```python
from build123d import *

# Parameters (mm, degrees)
SKETCH1_R           = 6
BOSS_EXTRUDE1_DEPTH = 91
SKETCH2_R           = 24.5
BOSS_EXTRUDE2_DEPTH = 4
SKETCH3_R           = 6
BOSS_EXTRUDE3_DEPTH = 3
BOSS_EXTRUDE4_DEPTH = 12
SKETCH5_R           = 6
BOSS_EXTRUDE5_DEPTH = 18
CHAMFER1_SIZE       = 0.9
SKETCH6_R           = 3
BOSS_EXTRUDE6_DEPTH = 20


with BuildPart() as part:
    # Sketch1 → Boss-Extrude1 (new body)
    with BuildSketch(Plane.XY):
        Circle(SKETCH1_R)
    extrude(amount=BOSS_EXTRUDE1_DEPTH)

    # Sketch2 → Boss-Extrude2 (add)
    with BuildSketch(Plane.XY.offset(91)):
        Circle(SKETCH2_R)
    extrude(amount=BOSS_EXTRUDE2_DEPTH)

    # Sketch3 → Boss-Extrude3 (add)
    with BuildSketch(Plane.XY.offset(95)):
        Circle(SKETCH3_R)
    extrude(amount=BOSS_EXTRUDE3_DEPTH)

    # Sketch4 → Boss-Extrude4 (add)
    with BuildSketch(Plane.XY.offset(98)):
        with BuildLine():
            Line((6, 5.291502622), (6, -5.291502622))
            ThreePointArc((6, -5.291502622), (0, -8), (-6, -5.291502622))
            Line((-6, -5.291502622), (-6, 5.291502622))
            ThreePointArc((-6, 5.291502622), (0, 8), (6, 5.291502622))
        make_face()
    extrude(amount=BOSS_EXTRUDE4_DEPTH)

    # Sketch5 → Boss-Extrude5 (add)
    with BuildSketch(Plane.XY.offset(110)):
        Circle(SKETCH5_R)
    extrude(amount=BOSS_EXTRUDE5_DEPTH)

    # Chamfer1
    chamfer1_edges = [part.edges().sort_by_distance(p)[0] for p in [
        (-6, 0, 0),
        (-6, 0, 128),
    ]]
    chamfer(chamfer1_edges, length=CHAMFER1_SIZE)

    # Sketch6 → Boss-Extrude6 (add)
    with BuildSketch(Plane.XY.offset(95)):
        with Locations((20, 0)):
            Circle(SKETCH6_R)
    extrude(amount=BOSS_EXTRUDE6_DEPTH)


solid = part.part
```
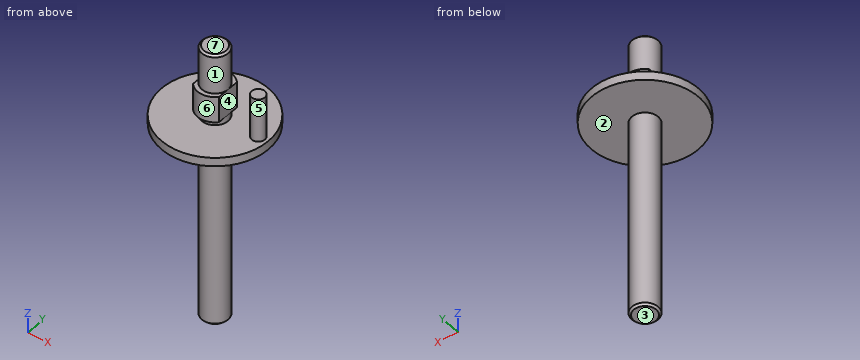
Source: CAD feature listing. Evaluate the final solid. Frame: model axes, mm. Face numbers are marked on the shaded views. A direction names the side the tool comes from. Coordinates: 2 decimals unless noted, no trailing zeros. Order: outer loops, then holes, each group sorted by start corner. A loop starts at its lowest first (then second) coordinate and runs counter-clockwise, first axis right, second up. Notation, with made-up numbers: (1, 39.5) - (26, 39.5) arc R16 cw to (26, 58.5) - close; hole circle Ø9 at (68, 56.5). An arc over 180 degrees is marked (long way). One line per item, written item: value.
1) Reachability of the marked faces 1, 2 and 3 from +Z, -Z, +X, -X, +Y, -Y: full face, straight path, thin tool, end or side. Return the list, or none.
Computed values:
face 1: +Z
face 2: -Z
face 3: -Z, +X, -X, +Y, -Y
2) Cut plane B-B on z = 79.5. Output: boundary loops of the cut face in (x, y).
Computed values:
outline: circle Ø12 at (0, 0)
3) Mould query, pull axis X, two halves, no side actions, for the marked faces 4, 5, 6 and 7. Classes: released by +X, released by -X, zero draft, split by the parting line, or undercut.
Computed values:
face 4: undercut
face 5: undercut
face 6: split by the parting line
face 7: zero draft
4) Cut plane C-C on y = -20. Output: boundary loops of the cut face in (x, z).
Computed values:
outline: (-14.15, 91) - (14.15, 91) - (14.15, 95) - (-14.15, 95) - close
5) Cut plane A-A on x = 0. Output: boundary loops of the cut face in (y, z), plus the area to 3 significant figures.
Computed values:
outline: (-24.5, 91) - (-6, 91) - (-6, 0.9) - (-5.1, 0) - (5.1, 0) - (6, 0.9) - (6, 91) - (24.5, 91) - (24.5, 95) - (6, 95) - (6, 98) - (8, 98) - (8, 110) - (6, 110) - (6, 127.1) - (5.1, 128) - (-5.1, 128) - (-6, 127.1) - (-6, 110) - (-8, 110) - (-8, 98) - (-6, 98) - (-6, 95) - (-24.5, 95) - close
area: 1,730 mm^2
6) Ray query, line 1 (Z direction, x = -5.5, y = -12.5); line 2 (X direction, y = -0.5, z = 96.5); line 3 (Z direction, x = -5, y = -4.5). Return the intervals inside material, ascending. Write a range as [from, to].
Computed values:
line 1: z = [91, 95]
line 2: x = [-5.98, 5.98], [17.04, 22.96]
line 3: z = [91, 95], [98, 110]
7) Contact query for flat-ended pins moving along their axis: pin 1 (1 mm diameter, centred on x = -9.5, y = -15, fed in from +Z); pin 2 (3 mm diameter, centred on y = 2, z = 107, fed in from -X); pin 3 (1.5 mm diameter, centred on x = -14, y = -18.5, fed in from -Z). Output: stop coordinate, or through.
Computed values:
pin 1: stops at z = 95
pin 2: stops at x = -6
pin 3: stops at z = 91
8) Cut plane D-D on x = 20. Output: boundary loops of the cut face in (y, z).
Computed values:
outline: (-14.15, 91) - (14.15, 91) - (14.15, 95) - (3, 95) - (3, 115) - (-3, 115) - (-3, 95) - (-14.15, 95) - close
